Can you work these out from the drawing? Everything is in mm from the part's minimum corner. Give positions to 0.01 mm unless a question says otherwise; leave off trailing zeros. Write each loop counter-clockwise with the first axis right and the second up, starting at its lowest first coordinate (ties: lowest second). Pieces come first, ordered by that corner, then holes. Notation, with made-up numbers: (24, -11) -> (60, -11) arc R11 ccw to (60, -5) -> close; hole circle Ø10 at (-25, 62.25). An arc over 180 degrees is marked (long way). Use one line per item in the form item = value.
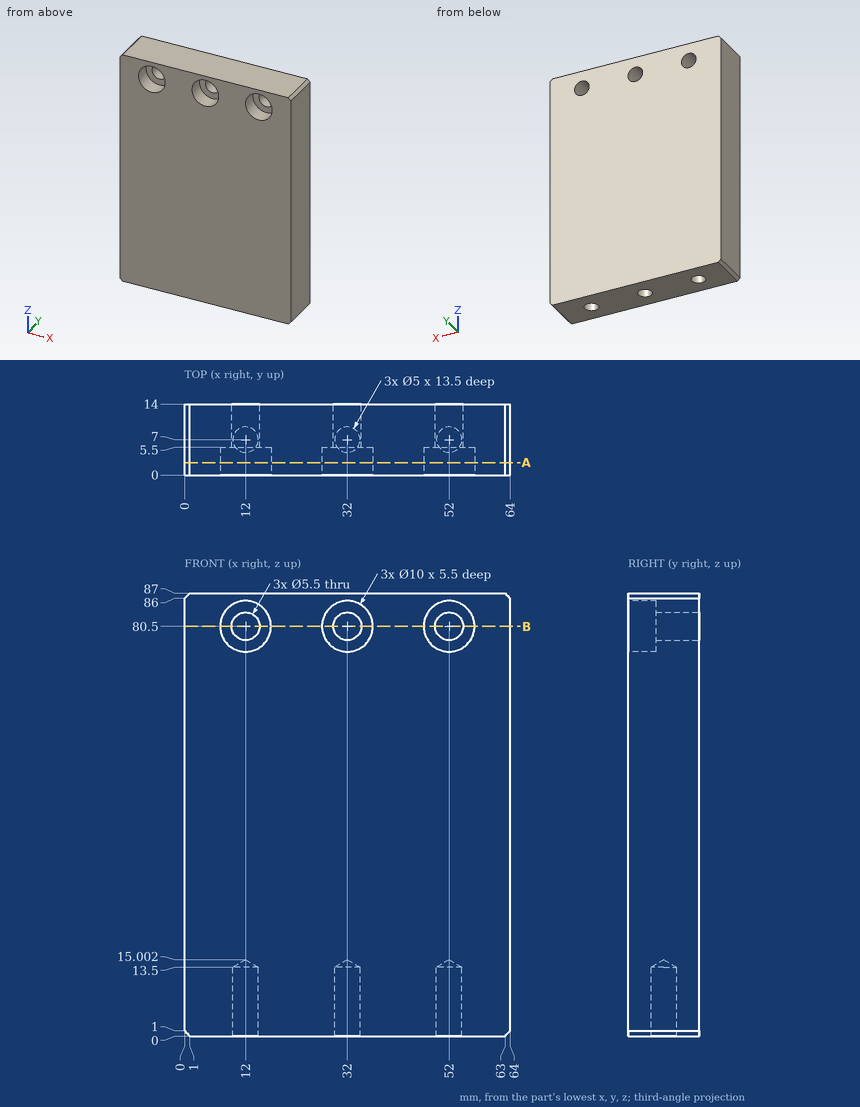
Q1. Will these pins go through, and if not, where does the flat tip stop? pin 1 Ø3.5 at (x, z) = (32, 80.5) entering from +Y; pin 2 Ø5 at (x, z) = (31, 79) entering from -Y; pin 3 Ø4.5 at (x, y) = (12, 7) entering from -Z.
Result set:
pin_1 = through
pin_2 = 5.5
pin_3 = 13.65
Q2. I want a section at B-B, the plane z = 80.5. Write out the boundary of the cut face in (x, y), and give its area (3 significant figures).
Result set:
outline = (0, 0) -> (7, 0) -> (7, 5.5) -> (9.25, 5.5) -> (9.25, 14) -> (0, 14) -> close; (14.75, 5.5) -> (17, 5.5) -> (17, 0) -> (27, 0) -> (27, 5.5) -> (29.25, 5.5) -> (29.25, 14) -> (14.75, 14) -> close; (34.75, 5.5) -> (37, 5.5) -> (37, 0) -> (47, 0) -> (47, 5.5) -> (49.25, 5.5) -> (49.25, 14) -> (34.75, 14) -> close; (54.75, 5.5) -> (57, 5.5) -> (57, 0) -> (64, 0) -> (64, 14) -> (54.75, 14) -> close
area = 591 mm2
Q3. I want a section at A-A, the plane y = 2.5. Write out the boundary of the cut face in (x, z).
Result set:
outline = (0, 1) -> (1, 0) -> (63, 0) -> (64, 1) -> (64, 86) -> (63, 87) -> (1, 87) -> (0, 86) -> close; hole circle Ø10 at (12, 80.5); hole circle Ø10 at (32, 80.5); hole circle Ø10 at (52, 80.5)
Q4. If I drill on line 1 along X through (y, z) = (10.25, 80.5); line 2 along Y through (x, z) = (52, 5.25); line 3 along Z through (x, y) = (32, 1.6), over which ranges is the centre line in solid material (lowest first)? Write a range as from..to.
Result set:
line_1 = 0..9.25, 14.75..29.25, 34.75..49.25, 54.75..64
line_2 = 0..4.5, 9.5..14
line_3 = 0..75.5, 85.5..87
